from build123d import *

# Parameters (mm, degrees)
SHELL1_T           = -2
SKETCH2_R          = 60
CUT_EXTRUDE1_DEPTH = 50
SKETCH3_R          = 5
CUT_EXTRUDE2_DEPTH = 50


with BuildPart() as part:
    # Sketch1 → Revolve1 (revolve)
    with BuildSketch(Plane(origin=(0, 0, 0), x_dir=(1, 0, 0), z_dir=(0, 1, 0)), mode=Mode.PRIVATE) as revolve1_sk:
        Polygon((0, 0), (0, 157.5), (30, 157.5), (30, 120), (40, 110), (40, 0), align=None)
    revolve(revolve1_sk.sketch.rotate(Axis((0, 0, 0), (1, 0, 0)), 180), axis=Axis((0, 0, 0), (1, 0, 0)))

    # Shell1
    shell1_openings = [part.faces().sort_by_distance(p)[0] for p in [
        (0, 0, 0),
    ]]
    offset(amount=SHELL1_T, openings=shell1_openings, kind=Kind.INTERSECTION)

    # Sketch2 → Cut-Extrude1 (cut)
    with BuildSketch(Plane(origin=(40, 0, 0), x_dir=(0, 0, -1), z_dir=(1, 0, 0))):
        Circle(SKETCH2_R)
    extrude(amount=-CUT_EXTRUDE1_DEPTH, mode=Mode.SUBTRACT)

    # Sketch3 → Cut-Extrude2 (cut)
    with BuildSketch(Plane(origin=(30, 0, 0), x_dir=(0, 0, -1), z_dir=(1, 0, 0))):
        with Locations((0, 135)):
            Circle(SKETCH3_R)
        with Locations((116.913429511, 67.5)):
            Circle(SKETCH3_R)
        with Locations((116.913429511, -67.5)):
            Circle(SKETCH3_R)
        with Locations((0, -135)):
            Circle(SKETCH3_R)
        with Locations((-116.913429511, -67.5)):
            Circle(SKETCH3_R)
        with Locations((-116.913429511, 67.5)):
            Circle(SKETCH3_R)
    extrude(amount=-CUT_EXTRUDE2_DEPTH, mode=Mode.SUBTRACT)


solid = part.part
The listing builds one solid part. Answer for the finished solid, in the listing's coordinates (mm). A direction names the side the tool comes from. Coordinates: 2 decimals unless noted, no trailing zeros. Order: outer loops, then holes, each group sorted by start corner. A loop starts at its lowest first (then second) coordinate and runs counter-clockwise, first axis right, second up. Notation, with made-up numbers: (-33, 5) -> (-20, 5) arc R23 ccw to (-20, 37) -> close; hole circle Ø4 at (31, 0.5). An arc over 180 degrees is marked (long way). Answer in a Markdown table with one row per item. Add a question column.
Item 1: Determine the mould class of faces 4 (the face through (14.196, -154.177, -20.243)), 5 (the face through (0, 104, -116)), 6 (the face through (39.51, 67.23, -87.68)) for opening direction Z: +Z half, -Z half, draft (parallel to the pull), parting line (faces both ways), or undercut.
Item 2: Find section A-A (x = 8.5). Write down the section's boundary in (y, z).
Item 3: Find the intervals of material crossed by L1, parallel to Y at x = 6.75, z = 0; L2, parallel to Z at x = 25, y = 3.5; L3, parallel to Y at x = 29.5, z = 0, in increasing order. Write a range as from..to.
Item 4: Which of the six approach directions +Z, -Z, +X, -X, +Y, -Y give full straight-line access (tool end or side, diameter ignored) to faces 1 (the face through (38, 47, 47)), 2 (the face through (29, -63.3, 114.2)), 3 (the face through (30, -106, -59))?
Item 5: Find section B-B (y = 135). Write down the section's boundary in (x, z), then the cut area to 3 significant figures.
Item 6: Each of these flat-tipped pins is pushed along its axis until it touches: P1, Ø4, axis at y = -61, z = 71, coming from the -X side; P2, Ø8, axis at y = -121, z = -47, coming from the +X side; P3, Ø1, axis at x = 10.5, z = 34, coming from the +Y side. Where does it stop, or does it pass through?
Item 7: Find section C-C (y = 67.5). State how many separate pieces and enclosed holes the cut face has, then the cut area to 3 significant figures.
Result set:
| question | item | result |
|---|---|---|
| 1 | face 4 | undercut |
| 1 | face 5 | draft |
| 1 | face 6 | parting line |
| 2 | outline | circle Ø315 at (0, 0); hole circle Ø311 at (0, 0) |
| 3 | L1 | y = -157.5..-155.5, 155.5..157.5 |
| 3 | L2 | z = -157.46..-155.46, 155.46..157.46 |
| 3 | L3 | y = -157.5..-140, -130..-117.67, 117.67..130, 140..157.5 |
| 4 | face 1 | -X |
| 4 | face 2 | +X, -X |
| 4 | face 3 | +X |
| 5 | outline | (0, -81.12) -> (30, -81.12) -> (30, -5) -> (28, -5) -> (28, -77.17) -> (0, -77.17) -> close; (0, 77.17) -> (28, 77.17) -> (28, 5) -> (30, 5) -> (30, 81.12) -> (0, 81.12) -> close |
| 5 | area | 526 mm² |
| 6 | P1 | stops at x = 38 |
| 6 | P2 | stops at x = 30 |
| 6 | P3 | stops at y = 153.9 |
| 7 | separate pieces | 3 |
| 7 | enclosed holes | 0 |
| 7 | area | 674 mm² |
